Input: part model. Units: mm. Frame: model coordinates. A direction names the side the tool comes from. Coordinates: 2 decimals unless noted, no trailing zeros. Write each loop counter-clockwise with the first axis right and the second up, starting at its lowest first coordinate (ties: lowest second). Pieces come first, ordered by that corner, then holes.
1) Section query C-C (x = -340). Output: boundary loops of the cut face in (y, z).
2) Section query A-A (z = -640). Output: boundary loops of the cut face in (x, y), then the cut area to 3 significant figures.
3) Pin query (flat end, axial travel): pin 1 Ø24 at (y, z) = (287.5, -356.5) entering from -X; pin 2 Ø24 at (x, z) = (497, -554.5) entering from +Y; pin 3 Ø24 at (y, z) = (261, -455) entering from +X. Return the tip coordinate at first contact, or that it passes through.
4) Set-up query: faces 4 (the flat face through (479, -320, -435)), 5 (the flat face through (440, -281, -435)), 6 (the flat face through (479, 240, -435)). Return all of +Z, -Z, +X, -X, +Y, -Y with unobstructed straight access to the full face (end or side cutting, diameter ignored); none if empty.
5) Line query: L1, parallel to Y at x = -485.5, z = -620; L2, parallel to Z at x = -303.5, y = -289.5; L3, parallel to X at y = -251, z = -606.5. Output: solid intervals per line, ascending.
6) Draft query along Y for faces 1 (the flat face through (479, -240, -435)), 2 (the flat face through (-520, -281, -435)), 3 (the flat face through (-479, 320, -435)). Return one class per face: pulls with the +Y half, pulls with the -Y half, needs draft (parallel to the pull), parting line crosses it, or undercut.
7) Section query B-B (y = 282). Output: boundary loops of the cut face in (x, z).
8) Section query D-D (y = 70.5). Output: boundary loops of the cut face in (x, z), then the cut area to 3 significant figures.
from build123d import *

# Parameters (mm, degrees)
SKETCH1_W               = 1200
SKETCH1_H               = 800
BOSS_EXTRUDE1_DEPTH     = 90
SKETCH2_W               = 80
SKETCH2_H               = 80
BOSS_EXTRUDE2_DEPTH     = 700
MIRROR2_COPY_1_SKETCH_W = 80
MIRROR2_COPY_1_SKETCH_H = 80
MIRROR2_COPY_1_DEPTH    = 700


with BuildPart() as part:
    # Sketch1 → Boss-Extrude1 (new body)
    with BuildSketch(Plane.XY):
        Rectangle(SKETCH1_W, SKETCH1_H)
    extrude(amount=-BOSS_EXTRUDE1_DEPTH)

    # Sketch2 → Boss-Extrude2 (add)
    with BuildSketch(Plane(origin=(0, 0, -90), x_dir=(-1, 0, 0), z_dir=(0, 0, -1))):
        with Locations((480, -280)):
            Rectangle(SKETCH2_W, SKETCH2_H)
    boss_extrude2 = extrude(amount=BOSS_EXTRUDE2_DEPTH)

    # Mirror1: Boss-Extrude2 across plane
    add(boss_extrude2.mirror(Plane.ZX))

    # Mirror2: Boss-Extrude2 across plane
    add(boss_extrude2.mirror(Plane(origin=(0, 0, 0), x_dir=(0, 0, 1), z_dir=(1, 0, 0))))

    # Mirror2 copy 1 sketch → Mirror2 copy 1 (add)
    with BuildSketch(Plane(origin=(0, 0, -90), x_dir=(1, 0, 0), z_dir=(0, 0, -1))):
        with Locations((480, -280)):
            Rectangle(MIRROR2_COPY_1_SKETCH_W, MIRROR2_COPY_1_SKETCH_H)
    extrude(amount=MIRROR2_COPY_1_DEPTH)


solid = part.part
Answer:
1. outline: (-400, -90) - (400, -90) - (400, 0) - (-400, 0) - close
2. outline: (-520, -320) - (-440, -320) - (-440, -240) - (-520, -240) - close; (-520, 240) - (-440, 240) - (-440, 320) - (-520, 320) - close; (440, -320) - (520, -320) - (520, -240) - (440, -240) - close; (440, 240) - (520, 240) - (520, 320) - (440, 320) - close
2. area: 25,600 mm2
3. pin 1: stops at x = -520
3. pin 2: stops at y = 320
3. pin 3: stops at x = 520
4. face 4: -Z, +X, -X, -Y
4. face 5: -Z, +Y, -Y
4. face 6: -Z, +X, -X
5. L1: y = -320 to -240, 240 to 320
5. L2: z = -90 to 0
5. L3: x = -520 to -440, 440 to 520
6. face 1: undercut
6. face 2: needs draft
6. face 3: pulls with the +Y half
7. outline: (-600, -90) - (-520, -90) - (-520, -790) - (-440, -790) - (-440, -90) - (440, -90) - (440, -790) - (520, -790) - (520, -90) - (600, -90) - (600, 0) - (-600, 0) - close
8. outline: (-600, -90) - (600, -90) - (600, 0) - (-600, 0) - close
8. area: 108,000 mm2
